Could you check a few things on this model? Use its own coordinates, in mm. Face numbers are marked on the shaded views. Give positions to 0.01 mm unless a question says otherwise; leave off trailing zeros. Order: outer loops, then holes, each group sorted by start corner. A loop starts at its lowest first (then second) coordinate and runs counter-clockwise, first axis right, second up.
(1) If I drill on probe 1 along X at (y, z) = (21.5, 76.5); probe 2 along Y at (x, z) = (47, 115); probe 3 along X at (y, z) = (25.5, 475.5), over which ranges is the centre line in solid material (lowest first)?
(2) If we mould it in two halves opening along X, with no side actions, what happens to the marked faces 1 and 2? For each: released by +X, released by -X, zero draft, split by the parting line, or undercut.
(3) Imagine slicing it at A-A, the plane y = 10. Write out the boundary of the cut face in (x, z), then the cut area to 3 significant figures.
(4) Imagine slicing it at C-C, the plane x = 29.5. Write out the boundary of the cut face in (y, z), then the cut area to 3 significant figures.
(5) Will these pins go through, and if not, where does the flat tip stop? pin 1 (12 mm diameter, centred on x = 56.5, z = 504, fed in from -Y); pin 2 (10 mm diameter, centred on x = 95, z = 552.5, fed in from +Y); pin 3 (3 mm diameter, centred on x = 67, y = 28.5, fed in from -Z).
(6) Imagine slicing it at B-B, the plane z = 478. Write out the boundary of the cut face in (x, y).
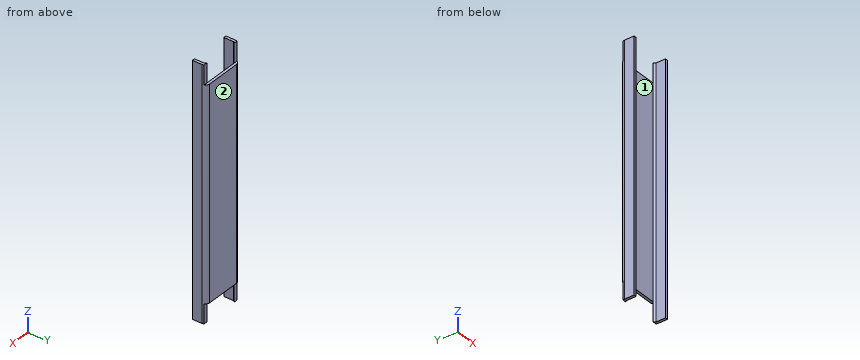
from build123d import *

# Parameters (mm, degrees)
BOSS_EXTRUDE1_DEPTH = 568
CUT_EXTRUDE1_DEPTH  = 44
CUT_EXTRUDE2_DEPTH  = 44


with BuildPart() as part:
    # Sketch1 → Boss-Extrude1 (new body)
    with BuildSketch(Plane.XY):
        with BuildLine():
            Line((0, 0), (0, 22))
            ThreePointArc((0, 22), (2.928932188, 29.071067812), (10, 32))
            Line((10, 32), (90, 32))
            ThreePointArc((90, 32), (97.071067812, 29.071067812), (100, 22))
            Line((100, 22), (100, 0))
            Line((100, 0), (94, 0))
            Line((94, 0), (94, 22))
            ThreePointArc((94, 22), (92.828427125, 24.828427125), (90, 26))
            Line((90, 26), (10, 26))
            ThreePointArc((10, 26), (7.171572875, 24.828427125), (6, 22))
            Line((6, 22), (6, 0))
            Line((6, 0), (0, 0))
        make_face()
    extrude(amount=BOSS_EXTRUDE1_DEPTH)

    # Sketch2 → Cut-Extrude1 (cut)
    with BuildSketch(Plane.XY.offset(568)):
        Polygon((-5.016704774, 26), (110.589606684, 26), (113.542758838, 46.117705453), (4.096772107, 46.117705453), (-12.020365044, 28.61582492), align=None)
    extrude(amount=-CUT_EXTRUDE1_DEPTH, mode=Mode.SUBTRACT)

    # Sketch3 → Cut-Extrude2 (cut)
    with BuildSketch(Plane(origin=(0, 0, 0), x_dir=(-1, 0, 0), z_dir=(0, 0, -1))):
        Polygon((-112.020365044, 26), (27.466483662, 26), (17.252014884, 45.492114728), (-47.890463774, 56.039795858), (-51.518866083, 56.039795858), (-99.243616331, 54.20535901), align=None)
    extrude(amount=-CUT_EXTRUDE2_DEPTH, mode=Mode.SUBTRACT)


solid = part.part
Answer block:
1. probe 1: x = 0 to 6, 94 to 100
1. probe 2: y = 26 to 32
1. probe 3: x = 0.63 to 8.06, 91.94 to 99.37
2. face 1: undercut
2. face 2: zero draft
3. outline: (0, 0) - (6, 0) - (6, 568) - (0, 568) - close; (94, 0) - (100, 0) - (100, 568) - (94, 568) - close
3. area: 6,820 mm2
4. outline: (26, 44) - (32, 44) - (32, 524) - (26, 524) - close
4. area: 2,880 mm2
5. pin 1: stops at y = 26
5. pin 2: stops at y = 26
5. pin 3: stops at z = 44
6. outline: (0, 0) - (6, 0) - (6, 22) arc R4 cw to (10, 26) - (90, 26) arc R4 cw to (94, 22) - (94, 0) - (100, 0) - (100, 22) arc R10 ccw to (90, 32) - (10, 32) arc R10 ccw to (0, 22) - close
